Design review of the part built by this model. Coordinates are the model's own, in mm. A direction names the side the tool comes from. Coordinates: 2 decimals unless noted, no trailing zeros. Write each loop counter-clockwise with the first axis right and the second up, starting at its lowest first coordinate (ties: lowest second). Pieces come first, ordered by that corner, then holes. Notation, with made-up numbers: M -1,-21 L 28,-21 A20 cw 28,2 Z; hole C -10.75,-27.75 d10. An arc over 180 degrees is marked long. One line per question, with ' | ' between items.
from build123d import *

# Parameters (mm, degrees)
SKETCH3_R           = 27.5
SKETCH3_W           = 20
SKETCH3_H           = 9
CUT_EXTRUDE1_DEPTH  = 130
SKETCH4_R           = 5
BOSS_EXTRUDE3_DEPTH = 28


with BuildPart() as part:
    # Sketch 1 → Revolve1 (revolve)
    with BuildSketch(Plane.XY, mode=Mode.PRIVATE) as revolve1_sk:
        Polygon((70, 75), (75, 75), (75, 95), (70, 95), (70, 115), (75, 115), (75, 130), (0, 130), (0, 0), (75, 0), (75, 15), (70, 15), (70, 35), (75, 35), (75, 55), (70, 55), align=None)
    revolve(revolve1_sk.sketch.rotate(Axis((0, 0, 0), (0, 1, 0)), 90), axis=Axis((0, 0, 0), (0, 1, 0)))

    # Sketch3 → Cut-Extrude1 (cut)
    with BuildSketch(Plane(origin=(0, 130, 0), x_dir=(1, 0, 0), z_dir=(0, 1, 0))):
        Circle(SKETCH3_R)
        with Locations((0, -27.5)):
            Rectangle(SKETCH3_W, SKETCH3_H)
    extrude(amount=-CUT_EXTRUDE1_DEPTH, mode=Mode.SUBTRACT)

    # Sketch4 → Boss-Extrude3 (add)
    with BuildSketch(Plane.XZ):
        with Locations(Location((0, -60, 0), (0, 0, 270))):
            Circle(SKETCH4_R)
        with Locations(Location((42.425, -42.427813696, 0), (0, 0, 270))):
            Circle(SKETCH4_R)
        with Locations(Location((-42.425, -42.427813696, 0), (0, 0, 270))):
            Circle(SKETCH4_R)
    extrude(amount=BOSS_EXTRUDE3_DEPTH)


solid = part.part
1. Take a section at A-A (y = 2.5). Write out the cut boundary in (x, z), then the cut area to 3 significant figures.
Answer sheet:
outline: C 0,0 d150; hole M -10,25.62 A27.5 ccw long 10,25.62 L 10,32 L -10,32 Z | area: 15,200 mm^2
2. Insertion check: pin 1 Ø12 at (x, z) = (-36.5, 11) entering from -Y; pin 2 Ø5 at (y, z) = (25.5, -4.5) entering from -X; pin 3 Ø5 at (x, y) = (-9, 1.5) entering from -Z. Each pin has a flat end and moves straight along its axis. Give the tip position at first contact, or say it passes through.
Answer sheet:
pin 1: y = 0 | pin 2: x = -69.97 | pin 3: z = -74.72
3. To check wall thickness, follow line 1 along Y through (x, z) = (53, 49); line 2 along X through (y, z) = (80, 0); line 3 along X through (y, z) = (71, 0). State the ranges of each line that lie inside material, in increasing order. Write a range as [from, to].
Answer sheet:
line 1: [0, 15], [35, 55], [75, 95], [115, 130] | line 2: [-75, -27.5], [27.5, 75] | line 3: [-70, -27.5], [27.5, 70]
4. Draft analysis for pull direction X (two halves, no side actions). For faces 6 (the face through (66.538, 85.14, -34.608)), 7 (the face through (10, 66, 29)), 8 (the face through (-10, 66, 29)), 9 (the face through (-42, -28, -42)), state which applies: pulls with the +X half, pulls with the -X half, needs draft (parallel to the pull), parting line crosses it, or undercut.
Answer sheet:
face 6: parting line crosses it | face 7: undercut | face 8: undercut | face 9: needs draft
5. Take a section at D-D (x = 55). Write out the cut boundary in (y, z).
Answer sheet:
outline: M 0,-50.99 L 15,-50.99 L 15,-43.3 L 35,-43.3 L 35,-50.99 L 55,-50.99 L 55,-43.3 L 75,-43.3 L 75,-50.99 L 95,-50.99 L 95,-43.3 L 115,-43.3 L 115,-50.99 L 130,-50.99 L 130,50.99 L 115,50.99 L 115,43.3 L 95,43.3 L 95,50.99 L 75,50.99 L 75,43.3 L 55,43.3 L 55,50.99 L 35,50.99 L 35,43.3 L 15,43.3 L 15,50.99 L 0,50.99 Z
6. Tool access review of faces 1 (the face through (43.927, -13.804, -47.197)), 2 (the face through (50, 115, 50)), 3 (the face through (0, 66, 32)), 4 (the face through (42, -28, -42)), 5 (the face through (32, 130, 1)): name each direction out of +Z, -Z, +X, -X, +Y, -Y from which nothing blocks a thin tool from reaching the whole face with its end or side.
Answer sheet:
face 1: -Y | face 2: none | face 3: +Y, -Y | face 4: +Z, -Z, +X, -X, -Y | face 5: +Z, -Z, +X, -X, +Y
